Check sheet for the drawn part. Datum: minimum x, y, z corner. Units: mm. A direction names the side the tool comes from. Give positions to 0.01 mm unless a question says otherwise; leave off trailing zeros. Order: outer loops, then holes, each group sorted by start corner. A loop starts at its lowest first (then second) coordinate and runs counter-clockwise, first axis right, second up.
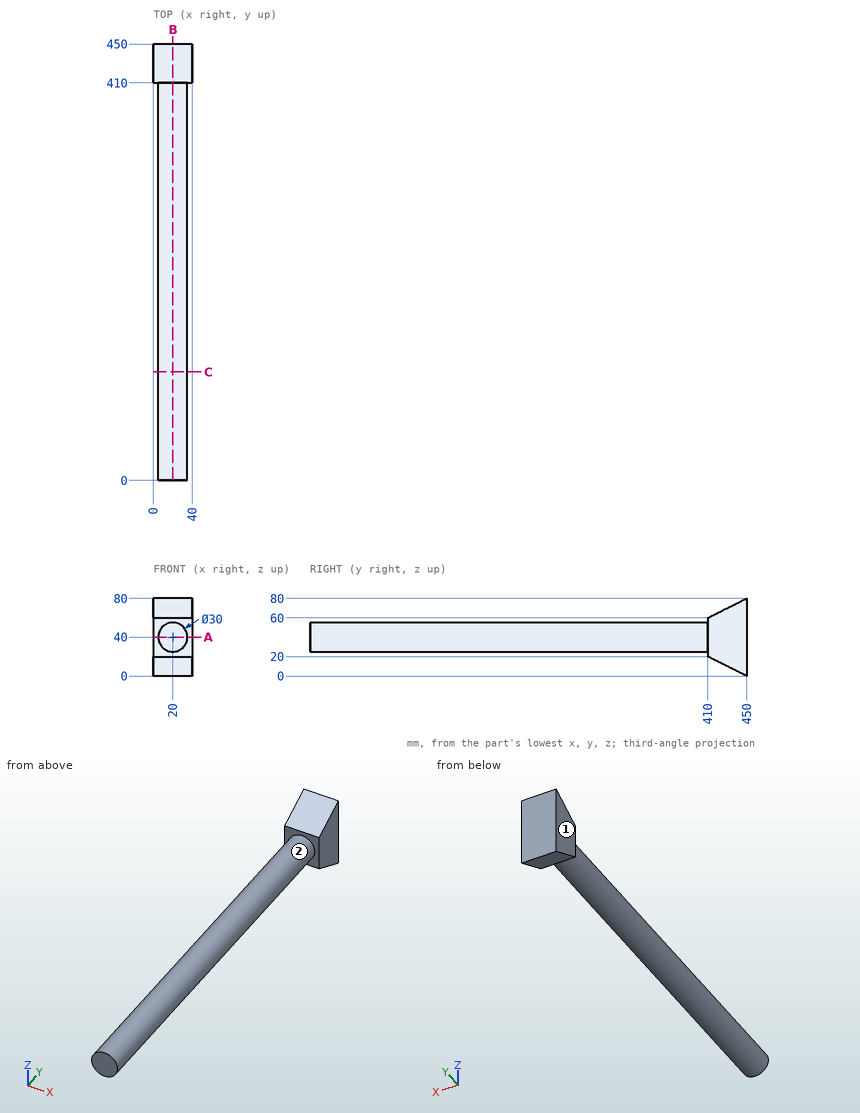
(1) Section check A-A, the plane z = 40. Enter the section's corners in (x, y).
Solved:
outline: (0, 410) - (5, 410) - (5, 0) - (35, 0) - (35, 410) - (40, 410) - (40, 450) - (0, 450) - close
(2) Section check B-B, the plane x = 20. Enter the section's corners in (y, z).
Solved:
outline: (0, 25) - (410, 25) - (410, 20) - (450, 0) - (450, 80) - (410, 60) - (410, 55) - (0, 55) - close
(3) Go/stop test with flat-tipped pins: pin 1 (1 mm diameter, centred on y = 256.5, z = 37, fed in from +X); pin 2 (2 mm diameter, centred on y = 244.5, z = 51, fed in from -X); pin 3 (8 mm diameter, centred on x = 28, z = 69.5, fed in from -Y). Record where each tip stops, or that it passes through.
Solved:
pin 1: stops at x = 34.79
pin 2: stops at x = 8.82
pin 3: stops at y = 421
(4) Set-up check for the marked faces 1 and 2: record each of +Z, -Z, +X, -X, +Y, -Y from which the full face is reachable in a straight line by a thin tool's end or side.
Solved:
face 1: +Z, -Z, -X, +Y, -Y
face 2: -Y
(5) Section check C-C, the plane y = 112. Enter the section's corners in (x, z), then the cut area to 3 significant figures.
Solved:
outline: circle Ø30 at (20, 40)
area: 707 mm2
(6) Scan lines: line 1 (Z direction, x = 20.5, y = 77.5); line 2 (Y direction, x = 8, z = 26); line 3 (X direction, y = 46, z = 31). Record each from-to range of solid material in increasing order.
Solved:
line 1: z = 25.01 to 54.99
line 2: y = 410 to 450
line 3: x = 8 to 32
